For this review, take the finished solid that the model builds, in its own axes (mm). A direction names the side the tool comes from. Give positions to 0.01 mm unless a question says otherwise; leave off trailing zeros. Loops run counter-clockwise (first coordinate to the right, second up) from the corner with the lowest first, then second, coordinate; pieces in that order, holes last. Notation, with made-up numbers: M 28.5,84.25 L 45.5,84.25 A26 ccw 45.5,117.25 Z; hole C 71.5,39.5 d4. An arc over 180 degrees is marked long. Use CSV: the item, a comma, the result in double quotes. Start each with the question number.
1. Insertion check: P1, Ø4, axis at x = 0, z = 10.5, coming from the +Y side; P2, Ø2, axis at x = 0, z = 85.5, coming from the -Y side; P3, Ø1.1, axis at y = 1.5, z = 36, coming from the -X side. Each pin has a flat end and moves straight along its axis. Give the tip position at first contact, or say it passes through.
2. Tool access review of faces 5 (the face through (-0.67, -2.226, 62.117)), 6 (the face through (0, -0.5, 37.5)): name each direction out of +Z, -Z, +X, -X, +Y, -Y from which nothing blocks a thin tool from reaching the whole face with its end or side.
3. Take a section at A-A, the plane z = 35.5. Write out the cut boundary in (x, y).
4. To check wall thickness, follow line 1 (Y direction, x = 5, z = 67.5); line 2 (Z direction, x = 1.25, y = 1.5); line 3 (X direction, y = 1.8, z = 10.5). State the ranges of each line that lie inside material, in increasing order. Write a range as [from, to].
5. Take a section at B-B, the plane z = 10. Write out the cut boundary in (x, y), and give its area (3 significant figures).
6. The part is to be moulded in two halves that separate along X. For faces 1 (the face through (-2.93, 1.78, 9.85)), 2 (the face through (-3.4, 4, 59.7)), 3 (the face through (1.18, -2.23, 34.21)), 4 (the face through (6, -1, 60)), say which applies: pulls with the +X half, pulls with the -X half, needs draft (parallel to the pull), parting line crosses it, or undercut.
from build123d import *

# Parameters (mm, degrees)
BOSS_EXTRUDE1_DEPTH = 121
SKETCH2_R           = 3
CUT_EXTRUDE1_DEPTH  = 4.5
SKETCH3_R           = 1.75
CUT_EXTRUDE2_DEPTH  = 122.232215191


with BuildPart() as part:
    # Sketch1 → Boss-Extrude1 (new body)
    with BuildSketch(Plane.XY):
        with BuildLine():
            Line((-5, 4), (5, 4))
            ThreePointArc((5, 4), (5.707106781, 3.707106781), (6, 3))
            Line((6, 3), (5, 2))
            Line((5, 2), (4, 2))
            Line((4, 2), (4, 1))
            Line((4, 1), (5, 1))
            Line((5, 1), (6, 0))
            Line((6, 0), (6, -3))
            ThreePointArc((6, -3), (5.707106781, -3.707106781), (5, -4))
            Line((5, -4), (-5, -4))
            ThreePointArc((-5, -4), (-5.707106781, -3.707106781), (-6, -3))
            Line((-6, -3), (-6, 0))
            Line((-6, 0), (-5, 1))
            Line((-5, 1), (-4, 1))
            Line((-4, 1), (-4, 2))
            Line((-4, 2), (-5, 2))
            Line((-5, 2), (-6, 3))
            ThreePointArc((-6, 3), (-5.707106781, 3.707106781), (-5, 4))
        make_face()
    extrude(amount=BOSS_EXTRUDE1_DEPTH)

    # Sketch2 → Cut-Extrude1 (cut)
    with BuildSketch(Plane(origin=(0, 4, 0), x_dir=(1, 0, 0), z_dir=(0, 1, 0))):
        with Locations(Location((0, -10.5, 0), (0, 0, 270))):
            Circle(SKETCH2_R)
        with Locations(Location((0, -35.5, 0), (0, 0, 270))):
            Circle(SKETCH2_R)
        with Locations(Location((0, -60.5, 0), (0, 0, 270))):
            Circle(SKETCH2_R)
        with Locations(Location((0, -85.5, 0), (0, 0, 270))):
            Circle(SKETCH2_R)
        with Locations(Location((0, -110.5, 0), (0, 0, 270))):
            Circle(SKETCH2_R)
    extrude(amount=-CUT_EXTRUDE1_DEPTH, mode=Mode.SUBTRACT)

    # Sketch3 → Cut-Extrude2 (cut, through all)
    with BuildSketch(Plane(origin=(0, -0.5, 0), x_dir=(1, 0, 0), z_dir=(0, 1, 0))):
        with Locations(Location((0, -35.5, 0), (0, 0, 270))):
            Circle(SKETCH3_R)
        with Locations(Location((0, -10.5, 0), (0, 0, 270))):
            Circle(SKETCH3_R)
        with Locations(Location((0, -60.5, 0), (0, 0, 270))):
            Circle(SKETCH3_R)
        with Locations(Location((0, -85.5, 0), (0, 0, 270))):
            Circle(SKETCH3_R)
        with Locations(Location((0, -110.5, 0), (0, 0, 270))):
            Circle(SKETCH3_R)
    extrude(amount=-CUT_EXTRUDE2_DEPTH, mode=Mode.SUBTRACT)


solid = part.part
Result set:
1,P1,"y = -0.5"
1,P2,"through"
1,P3,"x = -5.05"
2,face 5,"+Y, -Y"
2,face 6,"+Y"
3,outline,"M -6,-3 A1 ccw -5,-4 L -1.75,-4 L -1.75,-0.5 L -3,-0.5 L -3,4 L -5,4 A1 ccw -6,3 L -5,2 L -4,2 L -4,1 L -5,1 L -6,0 Z; M 1.75,-4 L 5,-4 A1 ccw 6,-3 L 6,0 L 5,1 L 4,1 L 4,2 L 5,2 L 6,3 A1 ccw 5,4 L 3,4 L 3,-0.5 L 1.75,-0.5 Z"
4,line 1,"[-4, 1], [2, 4]"
4,line 2,"[0, 7.77], [13.23, 32.77], [38.23, 57.77], [63.23, 82.77], [88.23, 107.77], [113.23, 121]"
4,line 3,"[-4, -3], [3, 4]"
5,outline,"M -6,-3 A1 ccw -5,-4 L -1.68,-4 L -1.68,-0.5 L -2.96,-0.5 L -2.96,4 L -5,4 A1 ccw -6,3 L -5,2 L -4,2 L -4,1 L -5,1 L -6,0 Z; M 1.68,-4 L 5,-4 A1 ccw 6,-3 L 6,0 L 5,1 L 4,1 L 4,2 L 5,2 L 6,3 A1 ccw 5,4 L 2.96,4 L 2.96,-0.5 L 1.68,-0.5 Z"
5,area,"50.8 mm2"
6,face 1,"undercut"
6,face 2,"needs draft"
6,face 3,"undercut"
6,face 4,"pulls with the +X half"
